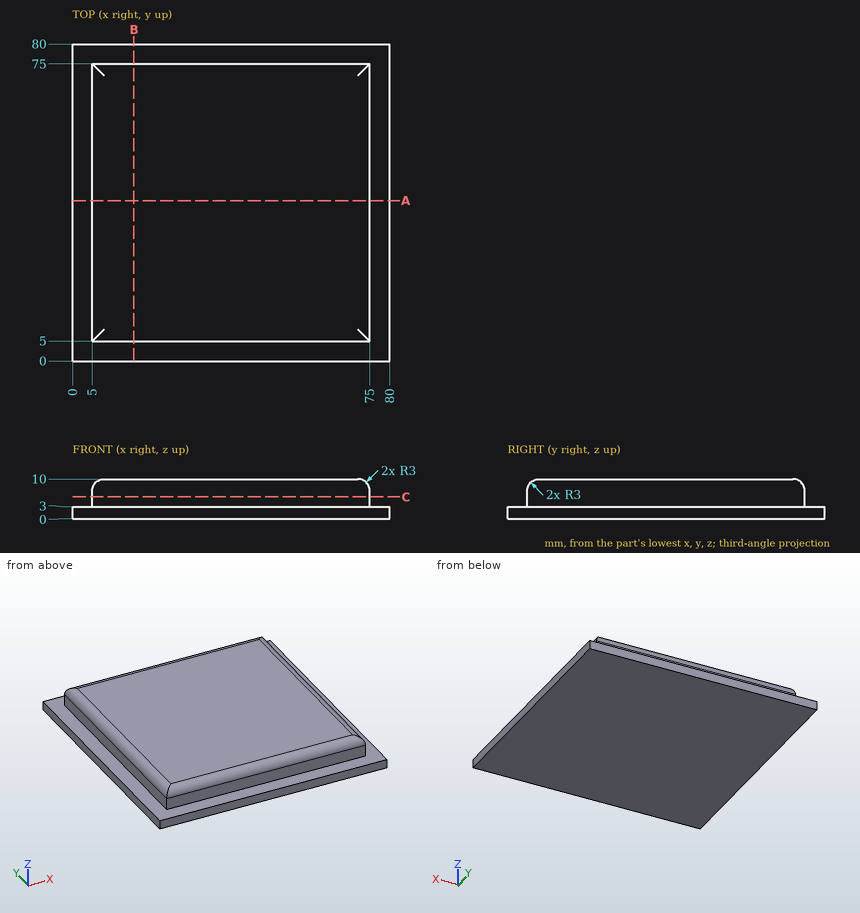
Can you work these out from the drawing? Everything is in mm from the part's minimum corner. Coordinates: 2 decimals unless noted, no trailing zeros. Write each loop counter-clockwise with the first axis right and the second up, starting at its lowest first coordinate (ties: lowest second). Pieces come first, ordered by that corner, then holes. Notation, with made-up numbers: (42, 15.25) -> (80, 15.25) arc R15 ccw to (80, 28.25) -> close; hole circle Ø6 at (35, 77). An arc over 180 degrees is marked (long way). Write each question's results on one line, items separated by ' | '. Start each with the question number.
Item 1: I'm going to push flat-ended pins straight in: P1, Ø1.2, axis at y = 57, z = 4.5, coming from the -X side; P2, Ø4.5, axis at x = 25, z = 5.5, coming from the +Y side; P3, Ø2, axis at y = 55.5, z = 5, coming from the +X side. Where does each tip first touch, or does it pass through?
Item 2: Please list where these lines run through material, in increasing order: probe 1 along Z at (x, y) = (75.5, 60); probe 2 along Y at (x, z) = (36, 7.25); probe 3 along X at (y, z) = (29.5, 5.5).
Item 3: If we section it at A-A, the plane y = 40.5: Write out the boundary of the cut face in (x, z).
Item 4: If we section it at C-C, the plane z = 5.5: Write out the boundary of the cut face in (x, y).
Answer block:
1) P1: x = 5 | P2: y = 75 | P3: x = 75
2) probe 1: 0 to 3 | probe 2: 5.01 to 74.99 | probe 3: 5 to 75
3) outline: (0, 0) -> (80, 0) -> (80, 3) -> (75, 3) -> (75, 7) arc R3 ccw to (72, 10) -> (8, 10) arc R3 ccw to (5, 7) -> (5, 3) -> (0, 3) -> close
4) outline: (5, 5) -> (75, 5) -> (75, 75) -> (5, 75) -> close
